```python
from build123d import *

# Parameters (mm, degrees)
FILLET1_R           = 2
SKETCH2_R           = 4
BOSS_EXTRUDE1_DEPTH = 10
FILLET2_R           = 2


with BuildPart() as part:
    # Sketch1 → Revolve1 (revolve)
    with BuildSketch(Plane.XY, mode=Mode.PRIVATE) as revolve1_sk:
        Polygon((30, 20), (30, 0), (0, 0), (0, 8), align=None)
    revolve(revolve1_sk.sketch.rotate(Axis((10.657678515, 0, 0), (1, 0, 0)), 90), axis=Axis((10.657678515, 0, 0), (1, 0, 0)))

    # Fillet1
    fillet1_edges = [part.edges().sort_by_distance(p)[0] for p in [
        (0, 0, -8),
    ]]
    fillet(fillet1_edges, radius=FILLET1_R)

    # Sketch2 → Boss-Extrude1 (add)
    with BuildSketch(Plane(origin=(30, 0, 0), x_dir=(0, 0, -1), z_dir=(1, 0, 0))):
        with Locations(Location((0, 0, 0), (0, 0, 180))):
            Circle(SKETCH2_R)
    extrude(amount=BOSS_EXTRUDE1_DEPTH)

    # Fillet2
    fillet2_edges = [part.edges().sort_by_distance(p)[0] for p in [
        (30, 0, -20),
    ]]
    fillet(fillet2_edges, radius=FILLET2_R)


solid = part.part
```
Part model, mm, in its own coordinate system. A direction names the side the tool comes from. Round coordinates to 2 decimals unless told otherwise and drop trailing zeros. Loops run counter-clockwise (first coordinate to the right, second up) from the corner with the lowest first, then second, coordinate; pieces in that order, holes last. Notation, with made-up numbers: (-14.5, -3) -> (-5.5, -3) arc R25 ccw to (-5.5, 9) -> close; hole circle Ø1 at (-12, 69.5). An arc over 180 degrees is marked (long way). Use a Markdown table: item, result.
1) Drop flat-ended pins along their axis: pin 1 Ø2 at (x, z) = (20, 6.5) entering from +Y; pin 2 Ø2 at (x, z) = (25.5, 4) entering from +Y; pin 3 Ø5 at (y, z) = (-7, -12.5) entering from +X; pin 4 Ø8 at (y, z) = (1, -4) entering from +X. Give the stop position or say it passes through.
The answers:
| item | result |
|---|---|
| pin 1 | stops at y = 15.22 |
| pin 2 | stops at y = 18.21 |
| pin 3 | stops at x = 30 |
| pin 4 | stops at x = 40 |
2) Cut at A-A, the plane y = 0. List the corners of the cut face in (x, z).
The answers:
| item | result |
|---|---|
| outline | (0, -6.65) arc R2 ccw to (1.26, -8.5) -> (27.26, -18.9) arc R2 ccw to (30, -17.05) -> (30, -4) -> (40, -4) -> (40, 4) -> (30, 4) -> (30, 17.05) arc R2 ccw to (27.26, 18.9) -> (1.26, 8.5) arc R2 ccw to (0, 6.65) -> close |
3) Cut at D-D, the plane x = 16. List the corners of the cut face in (y, z).
The answers:
| item | result |
|---|---|
| outline | circle Ø28.8 at (0, 0) |
4) Cut at C-C, the plane x = 37. List the corners of the cut face in (y, z).
The answers:
| item | result |
|---|---|
| outline | circle Ø8 at (0, 0) |
5) Probe line 1 (Z direction, x = 7.5, y = -8.5); line 2 (Z direction, x = 18, y = -11.5); line 3 (X direction, y = 12, z = -3.5). List the from-to ranges inside material, lowest first. Write a range as [from, to].
The answers:
| item | result |
|---|---|
| line 1 | z = [-6.98, 6.98] |
| line 2 | z = [-9.94, 9.94] |
| line 3 | x = [11.25, 30] |
6) Tool access for faces 1 (the cylindrical face through (34.93, 3.905, -0.867)), 2 (the conical face through (8.66, 11.19, -2.49)): list every direction of +Z, -Z, +X, -X, +Y, -Y with a clear straight run to the whole face (end or side of a thin tool).
The answers:
| item | result |
|---|---|
| face 1 | +X |
| face 2 | -X |
